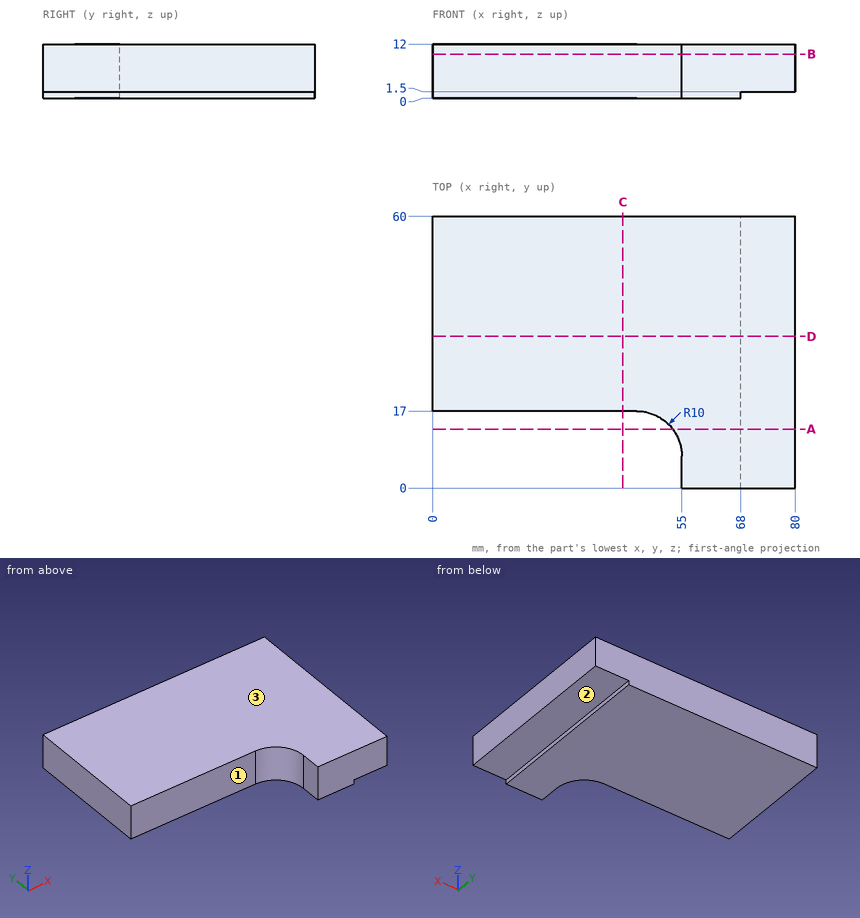
Source: three-view drawing plus pictorial views. Frame: mm from the lowest corner of the part. A direction names the side the tool comes from. Coordinates: 2 decimals unless noted, no trailing zeros. Write each loop counter-clockwise with the first axis right and the second up, starting at its lowest first coordinate (ties: lowest second). Pieces come first, ordered by that corner, then holes. Notation, with made-up numbers: (72.25, 56.25) -> (106.25, 56.25) arc R25 cw to (106.25, 95.25) -> close; hole circle Ø9 at (-14.5, 54.5). An arc over 180 degrees is marked (long way). Answer as a JSON object with one key per item and string values.
1. Section A-A on y = 13. Return the cut outline in (x, z), then the cut area to 3 significant figures.
Result set:
{"outline": "(53, 0) -> (68, 0) -> (68, 1.5) -> (80, 1.5) -> (80, 12) -> (53, 12) -> close", "area": "306 mm2"}
2. Section B-B on z = 9.75. Return the cut outline in (x, y), then the cut area to 3 significant figures.
Result set:
{"outline": "(0, 17) -> (45, 17) arc R10 cw to (55, 7) -> (55, 0) -> (80, 0) -> (80, 60) -> (0, 60) -> close", "area": "3,890 mm2"}
3. Access query for the marked faces 1, 2 and 3. Directions: +Z, -Z, +X, -X, +Y, -Y. A direction counts if a zero-diameter tool reaches every point of the face in a straight line with its end or side. Return the directions, or none.
Result set:
{"face 1": "+Z, -Z, -X, -Y", "face 2": "-Z, +X, +Y, -Y", "face 3": "+Z, +X, -X, +Y, -Y"}
4. Section C-C on x = 42. Return the cut outline in (y, z).
Result set:
{"outline": "(17, 0) -> (60, 0) -> (60, 12) -> (17, 12) -> close"}
5. First-contact query: P1, Ø6, axis at x = 25, z = 5.5, coming from the -Y side; P2, Ø1.6, axis at y = 19, z = 0.5, coming from the +X side; P3, Ø6, axis at x = 74.5, y = 42.5, coming from the -Z side. Flat tips, straight axial feed; report the tip coordinate or a pass-through.
Result set:
{"P1": "stops at y = 17", "P2": "stops at x = 68", "P3": "stops at z = 1.5"}
6. Material intervals for line 1 (Y direction, x = 9.5, z = 1.5); line 2 (Z direction, x = 75.5, y = 48); line 3 (X direction, y = 13, z = 11.25), sorted ascending. Write a range as from..to.
Result set:
{"line 1": "y = 17..60", "line 2": "z = 1.5..12", "line 3": "x = 53..80"}
7. Section D-D on y = 33.5. Return the cut outline in (x, z), then the cut area to 3 significant figures.
Result set:
{"outline": "(0, 0) -> (68, 0) -> (68, 1.5) -> (80, 1.5) -> (80, 12) -> (0, 12) -> close", "area": "942 mm2"}
